from build123d import *

# Parameters (mm, degrees)
BRACKET_PROFILE_SKETCH_R        = 5
BRACKET_PROFILE_SKETCH_R_2      = 11.5
BRACKET_BODY_DEPTH              = 37
SLOT_AND_CHANNEL_CUT_DEPTH      = 103.992718189
SLOT_AND_CHANNEL_CUT_DEPTH_BACK = 103.992718189
SLOT_AND_CHANNEL_SKETCH_W       = 27
SLOT_AND_CHANNEL_SKETCH_H       = 33
SLOT_AND_CHANNEL_SKETCH_H_2     = 77


with BuildPart() as part:
    # Bracket Profile Sketch → Bracket Body (new body)
    with BuildSketch(Plane.XY):
        with BuildLine():
            Line((-24.5, 63.5), (24.5, 63.5))
            ThreePointArc((24.5, 63.5), (33.692388155, 59.692388155), (37.5, 50.5))
            Line((37.5, 50.5), (37.5, -11.5))
            Line((37.5, -11.5), (24.374261359, -69.058361557))
            ThreePointArc((24.374261359, -69.058361557), (0, -88.5), (-24.374261359, -69.058361557))
            Line((-24.374261359, -69.058361557), (-37.5, -11.5))
            Line((-37.5, -11.5), (-37.5, 50.5))
            ThreePointArc((-37.5, 50.5), (-33.692388155, 59.692388155), (-24.5, 63.5))
        make_face()
        with Locations((24.5, 50.5)):
            Circle(BRACKET_PROFILE_SKETCH_R, mode=Mode.SUBTRACT)
        with Locations((-24.5, 50.5)):
            Circle(BRACKET_PROFILE_SKETCH_R, mode=Mode.SUBTRACT)
        with Locations((0, -63.5)):
            Circle(BRACKET_PROFILE_SKETCH_R_2, mode=Mode.SUBTRACT)
        with BuildLine():
            ThreePointArc((17.5, 7.226797096), (23.5, 13.226797096), (17.5, 19.226797096))
            Line((17.5, 19.226797096), (-17.5, 19.226797096))
            ThreePointArc((-17.5, 19.226797096), (-23.5, 13.226797096), (-17.5, 7.226797096))
            Line((-17.5, 7.226797096), (17.5, 7.226797096))
        make_face(mode=Mode.SUBTRACT)
    extrude(amount=BRACKET_BODY_DEPTH)

    # Slot and Channel Sketch → Slot and Channel Cut (cut, two sides: drawn at the far end of the back side and taken through both)
    with BuildSketch(Plane(origin=(0, 0, 0), x_dir=(0, 0, -1), z_dir=(1, 0, 0)).offset(-SLOT_AND_CHANNEL_CUT_DEPTH_BACK)):
        with Locations((-23.5, 47)):
            Rectangle(SLOT_AND_CHANNEL_SKETCH_W, SLOT_AND_CHANNEL_SKETCH_H)
        Polygon((0, 3), (0, 16), (-10, 16), (-10, 20.5), (-27, 20.5), (-27, -1.5), (-10, -1.5), (-10, 3), align=None)
        with Locations((-23.5, -50)):
            Rectangle(SLOT_AND_CHANNEL_SKETCH_W, SLOT_AND_CHANNEL_SKETCH_H_2)
    extrude(amount=SLOT_AND_CHANNEL_CUT_DEPTH + SLOT_AND_CHANNEL_CUT_DEPTH_BACK, mode=Mode.SUBTRACT)


solid = part.part
Check sheet for the modelled part. Datum: model origin and axes. Units: mm. A direction names the side the tool comes from. Give positions to 0.01 mm unless a question says otherwise; leave off trailing zeros. Loops run counter-clockwise (first coordinate to the right, second up) from the corner with the lowest first, then second, coordinate; pieces in that order, holes last. Notation, with made-up numbers: M 33,-35 L 79,-35 A24 cw 79,-12 Z; hole C 30,13.5 d2. An arc over 180 degrees is marked long. Return JSON: item names as keys, results as strings. Group by question number.
1. Cross-section at B-B on z = 17.5. Record the boundary of the cut face in (x, y), plus the area to 3 significant figures.
2. Tool access check on faces 4 (the cylindrical face through (-23.5, 13.36, 31.93)), 5 (the flat face through (-1, -11.5, 24)), 6 (the cylindrical face through (33.591, 59.793, 4.93)), 7 (the flat face through (-1, 20.5, 18)), 8 (the flat face through (30, 16, 5)). Record the directions out of +Z, -Z, +X, -X, +Y, -Y that give a thin tool (end or side, any length) a straight path to the whole face; none if there is none.
3. Mould release check, pull along Y, two halves, no side actions. Record for faces 1 (the cylindrical face through (0.471, -88.496, 4.93)), 2 (the flat face through (0, 19.227, 32)), 3 (the flat face through (1, -32, 0)): released by +Y, released by -Y, zero draft, split by the parting line, or undercut.
4. Cross-section at A-A on z = 6. Record the boundary of the cut face in (x, y).
5. Cross-section at C-C on x = -8. Record the boundary of the cut face in (y, z), plus the area to 3 significant figures.
6. Go/stop test with flat-tipped pins: pin 1 (11 mm diameter, centred on x = 28, z = 4.5, fed in from -Y); pin 2 (21.5 mm diameter, centred on x = -14.5, z = 26, fed in from -Y); pin 3 (13 mm diameter, centred on x = -24.5, y = 50.5, fed in from +Z). Record where each tip stops, or that it passes through.
7. Thickness scan on L1, parallel to X at y = 50.5, z = 4.75; L2, parallel to Y at x = -7.5, z = 16; L3, parallel to Y at x = -8.5, z = 35. Record the ranges inside material, lowest first.
8. Cross-section at D-D on y = -54.5. Record the boundary of the cut face in (x, z), plus the area to 3 significant figures.
Return value:
{
 "1": {"outline": "M -37.5,-11.5 L 37.5,-11.5 L 37.5,-1.5 L -37.5,-1.5 Z; M -37.5,20.5 L 37.5,20.5 L 37.5,30.5 L -37.5,30.5 Z", "area": "1,500 mm^2"},
 "2": {"face 4": "+Z, -Z", "face 5": "+Z, +X, -X, -Y", "face 6": "+Z, -Z, +X, +Y", "face 7": "+X, -X", "face 8": "-Z, +X, -X"},
 "3": {"face 1": "released by -Y", "face 2": "undercut", "face 3": "zero draft"},
 "4": {"outline": "M -37.5,-11.5 L -24.37,-69.06 A25 ccw 24.37,-69.06 L 37.5,-11.5 L 37.5,3 L -37.5,3 Z; M -37.5,16 L -22.82,16 A6 cw -17.5,19.23 L 17.5,19.23 A6 cw 22.82,16 L 37.5,16 L 37.5,50.5 A13 ccw 24.5,63.5 L -24.5,63.5 A13 ccw -37.5,50.5 Z; hole C -24.5,50.5 d10; hole C 0,-63.5 d23; hole C 24.5,50.5 d10"},
 "5": {"outline": "M -87.19,0 L -71.76,0 L -71.76,10 L -87.19,10 Z; M -55.24,0 L 3,0 L 3,10 L -1.5,10 L -1.5,27 L 7.23,27 L 7.23,37 L -11.5,37 L -11.5,10 L -55.24,10 Z; M 19.23,0 L 63.5,0 L 63.5,10 L 30.5,10 L 30.5,37 L 19.23,37 L 19.23,27 L 20.5,27 L 20.5,10 L 19.23,10 Z", "area": "1,820 mm^2"},
 "6": {"pin 1": "y = -74.4", "pin 2": "y = -11.5", "pin 3": "z = 10"},
 "7": {"L1": "-37.5 to -29.5, -19.5 to 19.5, 29.5 to 37.5", "L2": "-11.5 to -1.5, 20.5 to 30.5", "L3": "-11.5 to 7.23, 19.23 to 30.5"},
 "8": {"outline": "M -27.69,0 L -7.16,0 L -7.16,10 L -27.69,10 Z; M 7.16,0 L 27.69,0 L 27.69,10 L 7.16,10 Z", "area": "411 mm^2"}
}
